Could you check a few things on this model? Use its own coordinates, in mm. A direction names the side the tool comes from. Round coordinates to 2 decimals unless told otherwise and drop trailing zeros. Loops run counter-clockwise (first coordinate to the right, second up) from the corner with the lowest first, then second, coordinate; pieces in that order, holes last. Notation, with made-up numbers: (-2, 46.5) -> (7, 46.5) arc R10 cw to (7, 62.5) -> close; hole circle Ø6 at (22.5, -12). An arc over 180 degrees is marked (long way). One line per item, written item: value.
```python
from build123d import *

# Parameters (mm, degrees)
SKETCH_1_R      = 2.5
EXTRUDE_1_DEPTH = 20
EXTRUDE_2_DEPTH = 3


with BuildPart() as part:
    # 草图1 → 凸台-拉伸1 (new body)
    with BuildSketch(Plane.XY):
        Circle(SKETCH_1_R)
    extrude(amount=EXTRUDE_1_DEPTH)

    # 草图2 → 凸台-拉伸2 (add)
    with BuildSketch(Plane(origin=(0, 0, 0), x_dir=(-1, 0, 0), z_dir=(0, 0, -1))):
        Polygon((0.082884141, -4.04060188), (3.540705945, -1.948521168), (3.457821804, 2.092080712), (-0.082884141, 4.04060188), (-3.540705945, 1.948521168), (-3.457821804, -2.092080712), align=None)
    extrude(amount=EXTRUDE_2_DEPTH)


solid = part.part
```
Item 1: Will these pins go through, and if not, where does the flat tip stop? pin 1 Ø1.5 at (x, z) = (1.5, 7.5) entering from +Y; pin 2 Ø1.5 at (x, z) = (-1.5, 8) entering from -Y.
Output:
pin 1: stops at y = 2.38
pin 2: stops at y = -2.38
Item 2: If we section it at A-A on y = 0: List the corners of the cut face in (x, z) for me.
Output:
outline: (-3.5, -3) -> (3.5, -3) -> (3.5, 0) -> (2.5, 0) -> (2.5, 20) -> (-2.5, 20) -> (-2.5, 0) -> (-3.5, 0) -> close
Item 3: If we section it at D-D on y = 2.75: List the corners of the cut face in (x, z) for me.
Output:
outline: (-2.26, -3) -> (2.22, -3) -> (2.22, 0) -> (-2.26, 0) -> close
Item 4: If we mould it in two halves opening along X, with no side actions, what happens to faces 3 (the face through (-0.54, -2.44, 9.86)), 4 (the face through (-1.8, -3, -1.5)), 5 (the face through (1.8, 3, -1.5))? For each: released by +X, released by -X, zero draft, split by the parting line, or undercut.
Output:
face 3: split by the parting line
face 4: released by -X
face 5: released by +X
Item 5: If we section it at B-B on x = -1.75: List the corners of the cut face in (y, z) for me.
Output:
outline: (-3.03, -3) -> (3.03, -3) -> (3.03, 0) -> (1.79, 0) -> (1.79, 20) -> (-1.79, 20) -> (-1.79, 0) -> (-3.03, 0) -> close
Item 6: If we section it at C-C on z = 3.5: List the corners of the cut face in (x, y) for me.
Output:
outline: circle Ø5 at (0, 0)
Item 7: I need wall thicknesses on line 1 (Z direction, x = -2.25, y = 1.5); line 2 (X direction, y = 0.75, z = 5). Which ranges of each line are inside material? Lowest first, please. Write a range as from..to.
Output:
line 1: z = -3..0
line 2: x = -2.38..2.38
Item 8: For faces 1 (the face through (0, -3, 0)), 2 (the face through (1.712, -3.053, -1.479)), which set-ups out of +Z, -Z, +X, -X, +Y, -Y let a thin tool reach every point of the face, with its end or its side?
Output:
face 1: +Z
face 2: +Z, -Z, +X, -Y
